For this review, take the finished solid that the model builds, in its own axes (mm). Face numbers are marked on the shaded views. Round coordinates to 2 decimals unless told otherwise and drop trailing zeros. Order: outer loops, then holes, each group sorted by start corner. A loop starts at its lowest first (then second) coordinate and runs counter-clockwise, first axis right, second up. Notation, with made-up numbers: (6, -27.5) - (31, -27.5) arc R26 cw to (31, -7.5) - close; hole circle Ø5 at (42, 45). An arc over 180 degrees is marked (long way). One line per item, written item: value.
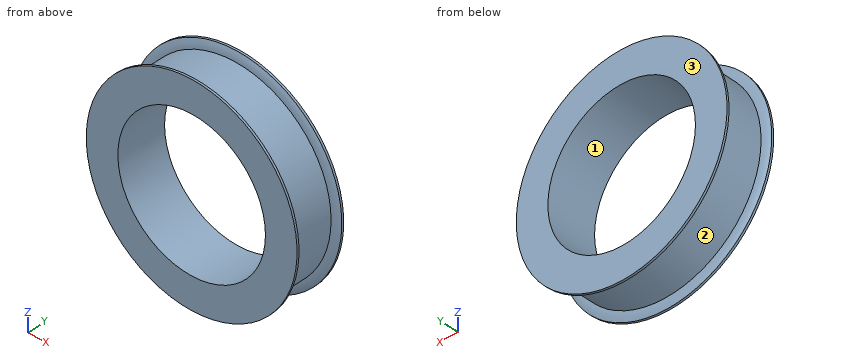
```python
from build123d import *


with BuildPart() as part:
    # Sketch1 → Revolve1 (revolve)
    with BuildSketch(Plane.XY, mode=Mode.PRIVATE) as revolve1_sk:
        Polygon((22.92, -5), (22.92, 5), (20, 5), (20, 6), (17.5, 6), (17.5, -6), (20, -6), (20, -5), align=None)
    revolve(revolve1_sk.sketch.rotate(Axis((0, 0, 0), (0, 1, 0)), 90), axis=Axis((0, 0, 0), (0, 1, 0)))

    # Sketch2 → Revolve2 (revolve)
    with BuildSketch(Plane.XY, mode=Mode.PRIVATE) as revolve2_sk:
        with BuildLine():
            Line((20, 5), (22.92, 5))
            ThreePointArc((22.92, 5), (23.9870538, 5.137456193), (25, 5.5))
            Line((25, 5.5), (25, 6))
            Line((25, 6), (20, 6))
            Line((20, 6), (20, 5))
        make_face()
        with BuildLine():
            Line((25, -5.5), (25, -6))
            Line((25, -6), (20, -6))
            Line((20, -6), (20, -5))
            Line((20, -5), (22.92, -5))
            ThreePointArc((22.92, -5), (23.9870538, -5.137456193), (25, -5.5))
        make_face()
    revolve(revolve2_sk.sketch.rotate(Axis((0, 0, 0), (0, 1, 0)), 90), axis=Axis((0, 0, 0), (0, 1, 0)))


solid = part.part
```
Item 1: Take a section at B-B (x = 0). Write out the cut boundary in (y, z).
Returned:
outline: (-6, -25) - (-5.5, -25) arc R5 ccw to (-5, -22.92) - (5, -22.92) arc R5 ccw to (5.5, -25) - (6, -25) - (6, -17.5) - (-6, -17.5) - close; (-6, 17.5) - (6, 17.5) - (6, 25) - (5.5, 25) arc R5 ccw to (5, 22.92) - (-5, 22.92) arc R5 ccw to (-5.5, 25) - (-6, 25) - close
Item 2: The part is to be moulded in two halves that separate along X. For the marked faces 1, 2 and 3, say which applies: +X half, -X half, draft (parallel to the pull), parting line (faces both ways), or undercut.
Returned:
face 1: undercut
face 2: parting line
face 3: draft
Item 3: For P1, Ø5, axis at x = 11.5, y = 3, coming from the +Z side; P2, Ø1.5, axis at x = 7.5, y = 1.5, coming from the +Z side; P3, Ø3, axis at x = 12.5, y = -0.5, coming from the -Z side, all flat-tipped, find the tip position at first contact; note any pin that passes through.
Returned:
P1: z = 22.33
P2: z = 21.9
P3: z = -20.11
Item 4: Wall thickness on line 1 (X direction, y = -1.75, z = 0); line 2 (Z direction, x = -14.5, y = -2.25); line 3 (Y direction, x = -17.5, z = 15): over which ranges is each line inside the solid? List them lowest first.
Returned:
line 1: -22.92 to -17.5, 17.5 to 22.92
line 2: -17.75 to -9.8, 9.8 to 17.75
line 3: -6 to -5, 5 to 6
Item 5: Take a section at A-A (z = 0). Write out the cut boundary in (x, y), plus the area to 3 significant figures.
Returned:
outline: (-25, -6) - (-17.5, -6) - (-17.5, 6) - (-25, 6) - (-25, 5.5) arc R5 ccw to (-22.92, 5) - (-22.92, -5) arc R5 ccw to (-25, -5.5) - close; (17.5, -6) - (25, -6) - (25, -5.5) arc R5 ccw to (22.92, -5) - (22.92, 5) arc R5 ccw to (25, 5.5) - (25, 6) - (17.5, 6) - close
area: 137 mm^2
Item 6: Take a section at C-C (y = -2.75). Write out the cut boundary in (x, z).
Returned:
outline: circle Ø45.84 at (0, 0); hole circle Ø35 at (0, 0)
